The model under review builds one solid part; all positions refer to its coordinate system, in mm. A direction names the side the tool comes from. Give positions to 0.01 mm unless a question says otherwise; leave off trailing zeros. Write each loop counter-clockwise with the first axis right and the second up, starting at its lowest first coordinate (ties: lowest second). Pieces come first, ordered by that corner, then holes. Notation, with made-up numbers: (13.25, -32.75) - (23.25, -32.75) arc R17 ccw to (23.25, 0.25) - close; hole circle Ø1 at (74.25, 2). An arc over 180 degrees is marked (long way). Write item = value, one per line.
```python
from build123d import *

# Parameters (mm, degrees)
SKETCH2_W           = 204
SKETCH2_H           = 28
BOSS_EXTRUDE1_DEPTH = 34
CHAMFER1_SIZE       = 20


with BuildPart() as part:
    # Sketch1 → Revolve1 (revolve)
    with BuildSketch(Plane.XY, mode=Mode.PRIVATE) as revolve1_sk:
        Polygon((0, 0), (0, 15), (145, 15), (145, 8), (165, 8), (165, 0), align=None)
    revolve(revolve1_sk.sketch.rotate(Axis((0, 0, 0), (1, 0, 0)), 90), axis=Axis((0, 0, 0), (1, 0, 0)))

    # Sketch2 → Boss-Extrude1 (add)
    with BuildSketch(Plane.ZY):
        Rectangle(SKETCH2_W, SKETCH2_H)
    extrude(amount=BOSS_EXTRUDE1_DEPTH)

    # Chamfer1
    chamfer1_edges = [part.edges().sort_by_distance(p)[0] for p in [
        (-34, 0, -102),
        (-34, 0, 102),
    ]]
    chamfer(chamfer1_edges, length=CHAMFER1_SIZE)


solid = part.part
```
1. Take a section at D-D on x = -18. Give the boundary of the cut face in (y, z), and give its area (3 significant figures).
Findings below:
outline = (-14, -98) - (14, -98) - (14, 98) - (-14, 98) - close
area = 5,490 mm²
2. Take a section at C-C on x = 137.5. Give the boundary of the cut face in (y, z), and give its area (3 significant figures).
Findings below:
outline = circle Ø30 at (0, 0)
area = 707 mm²
3. For line 1 (X direction, y = 8, z = 51); line 2 (X direction, y = 8.5, z = 0); line 3 (Y direction, x = -20, z = -21), list the stretches that pass through material, from the lowest coordinate up. Write a range as from..to.
Findings below:
line_1 = -34..0
line_2 = -34..145
line_3 = -14..14
4. Take a section at B-B on z = 0. Give the boundary of the cut face in (x, y), and give its area (3 significant figures).
Findings below:
outline = (-34, -14) - (0, -14) - (0, -15) - (145, -15) - (145, -8) - (165, -8) - (165, 8) - (145, 8) - (145, 15) - (0, 15) - (0, 14) - (-34, 14) - close
area = 5,620 mm²
5. Insertion check: P1, Ø10, axis at x = -11, z = -13.5, coming from the -Y side; P2, Ø1, axis at x = 132, y = 7, coming from the -Z side; P3, Ø10, axis at x = 15.5, y = -9, coming from the +Z side. Each pin has a flat end and moves straight along its axis. Give the tip position at first contact, or say it passes through.
Findings below:
P1 = -14
P2 = -13.52
P3 = 14.46
6. Take a section at A-A on y = 0. Give the boundary of the cut face in (x, z).
Findings below:
outline = (-34, -82) - (-14, -102) - (0, -102) - (0, -15) - (145, -15) - (145, -8) - (165, -8) - (165, 8) - (145, 8) - (145, 15) - (0, 15) - (0, 102) - (-14, 102) - (-34, 82) - close
7. Machinability: for faces 1 (the flat face through (-34, 0, -1)), 2 (the flat face through (145, 6, 6)), which of the approach directions +Z, -Z, +X, -X, +Y, -Y give a long, thin tool a straight path to every point of the face, cutting with its end or side? Answer none if there is none.
Findings below:
face_1 = +Z, -Z, -X, +Y, -Y
face_2 = +X
